from build123d import *

# Parameters (mm, degrees)
M4_TAPPED_HOLE1_D     = 3.3
M4_TAPPED_HOLE1_DEPTH = 8.1
M4_TAPPED_HOLE1_TIP   = 0.991420021
SKETCH3_R             = 1.5
CUT_EXTRUDE1_DEPTH    = 8
M3_TAPPED_HOLE2_D     = 2.5
M3_TAPPED_HOLE2_DEPTH = 7.5
M3_TAPPED_HOLE2_TIP   = 0.751075774
CHAMFER1_SIZE         = 0.5
M3_TAPPED_HOLE3_D     = 2.5
M3_TAPPED_HOLE3_DEPTH = 7.5
M3_TAPPED_HOLE3_TIP   = 0.751075774
SKETCH9_R             = 1.5
CUT_EXTRUDE2_DEPTH    = 8


with BuildPart() as part:
    # Sketch1 → Revolve1 (revolve)
    with BuildSketch(Plane.XY, mode=Mode.PRIVATE) as revolve1_sk:
        Polygon((0, 0), (-7.5, 0), (-7.5, -39), (-5, -39), (-5, -136.5), (0, -136.5), align=None)
    revolve(revolve1_sk.sketch.rotate(Axis((0, 0, 0), (0, -1, 0)), 270), axis=Axis((0, 0, 0), (0, -1, 0)))

    # M4 Tapped Hole1
    with Locations(Plane.ZX):
        with Locations((0, 0)):
            Hole(M4_TAPPED_HOLE1_D / 2, depth=M4_TAPPED_HOLE1_DEPTH)
            with Locations((0, 0, -(M4_TAPPED_HOLE1_DEPTH + M4_TAPPED_HOLE1_TIP / 2))):  # 118° drill point
                Cone(0, M4_TAPPED_HOLE1_D / 2, M4_TAPPED_HOLE1_TIP, mode=Mode.SUBTRACT)

    # Sketch3 → Cut-Extrude1 (cut, symmetric)
    with BuildSketch(Plane.XY):
        with Locations((0, -10)):
            Circle(SKETCH3_R)
    extrude(amount=CUT_EXTRUDE1_DEPTH, both=True, mode=Mode.SUBTRACT)

    # M3 Tapped Hole2
    with Locations(Plane(origin=(0, -136.5, 0), x_dir=(0, 0, -1), z_dir=(0, -1, 0))):
        with Locations((0, 0)):
            Hole(M3_TAPPED_HOLE2_D / 2, depth=M3_TAPPED_HOLE2_DEPTH)
            with Locations((0, 0, -(M3_TAPPED_HOLE2_DEPTH + M3_TAPPED_HOLE2_TIP / 2))):  # 118° drill point
                Cone(0, M3_TAPPED_HOLE2_D / 2, M3_TAPPED_HOLE2_TIP, mode=Mode.SUBTRACT)

    # Chamfer1
    chamfer1_edges = [part.edges().sort_by_distance(p)[0] for p in [
        (0, -136.5, -5),
        (0, -39, -7.5),
        (0, 0, -7.5),
    ]]
    chamfer(chamfer1_edges, length=CHAMFER1_SIZE)

    # M3 Tapped Hole3
    with Locations(Plane(origin=(-7.5, -10, 0), x_dir=(0, 0, -1), z_dir=(-1, 0, 0))):
        with Locations((0, 0)):
            Hole(M3_TAPPED_HOLE3_D / 2, depth=M3_TAPPED_HOLE3_DEPTH)
            with Locations((0, 0, -(M3_TAPPED_HOLE3_DEPTH + M3_TAPPED_HOLE3_TIP / 2))):  # 118° drill point
                Cone(0, M3_TAPPED_HOLE3_D / 2, M3_TAPPED_HOLE3_TIP, mode=Mode.SUBTRACT)

    # Sketch9 → Cut-Extrude2 (cut, symmetric)
    with BuildSketch(Plane.XY):
        with Locations((0, -109)):
            Circle(SKETCH9_R)
    extrude(amount=CUT_EXTRUDE2_DEPTH, both=True, mode=Mode.SUBTRACT)


solid = part.part
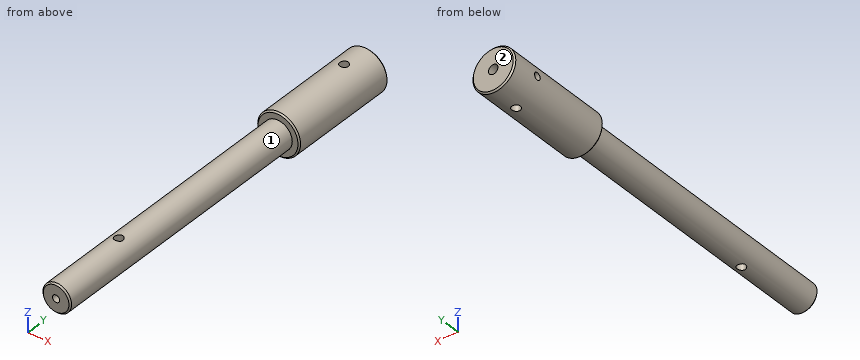
For this review, take the finished solid that the model builds, in its own axes (mm). Face numbers are marked on the shaded views. A direction names the side the tool comes from. Give positions to 0.01 mm unless a question says otherwise; leave off trailing zeros. Order: outer loops, then holes, each group sorted by start corner. A loop starts at its lowest first (then second) coordinate and runs counter-clockwise, first axis right, second up. Notation, with made-up numbers: (-24, 54) - (32, 54) arc R29 cw to (32, 78) - close; hole circle Ø4 at (57.5, -18). An arc over 180 degrees is marked (long way). Answer as a JSON object with one key per item and string values. Group by question number.
Item 1: Take a section at B-B on y = -94. Give the boundary of the cut face in (x, z), and give its area (3 significant figures).
Item 2: Take a section at A-A on y = -10. Give the boundary of the cut face in (x, z), and give its area (3 significant figures).
Item 3: Wall thickness on line 1 along X through (y, z) = (-132, 0); line 2 along Y through (x, z) = (0, 0); line 3 along Y through (x, z) = (-0.5, -4.25): over which ranges is each line inside the solid? List them lowest first.
Item 4: Machinability: for the marked faces 1 and 2, which of the approach directions +Z, -Z, +X, -X, +Y, -Y give a long, thin tool a straight path to every point of the face, cutting with its end or side? Answer none if there is none.
Item 5: Clearance check with flat-ended pins moving along their axes: pin 1 Ø3 at (x, z) = (0, 0) entering from -Y; pin 2 Ø5 at (x, y) = (3.5, -104.5) entering from -Z; pin 3 Ø1.8 at (x, y) = (0, -109) entering from +Z; pin 4 Ø3 at (x, z) = (0, 0) entering from +Y. State where each tip first meets the part, or that it passes through.
Reported:
{
 "1": {"outline": "circle Ø10 at (0, 0)", "area": "78.5 mm^2"},
 "2": {"outline": "(-7.4, -1.25) arc R7.5 ccw to (-1.5, -7.35) - (-1.5, -1.25) - close; (-7.4, 1.25) - (-1.5, 1.25) - (-1.5, 7.35) arc R7.5 ccw to start; (1.5, -7.35) arc R7.5 ccw to (1.5, 7.35) - close", "area": "117 mm^2"},
 "3": {"line 1": "-5 to -1.25, 1.25 to 5", "line 2": "-128.25 to -110.5, -107.5 to -11.5", "line 3": "-136.5 to -110.41, -107.59 to -11.41, -8.59 to 0"},
 "4": {"face 1": "-Y", "face 2": "+Z, -Z, +X, -X, +Y"},
 "5": {"pin 1": "y = -136.5", "pin 2": "z = -4.9", "pin 3": "through", "pin 4": "y = -8.19"}
}
